Could you check a few things on this model? Use its own coordinates, in mm. Give positions to 0.01 mm unless a question says otherwise; leave off trailing zeros. Order: outer loops, then holes, each group sorted by start corner. A loop starts at its lowest first (then second) coordinate and runs counter-clockwise, first axis right, second up.
(1) If I drill on probe 1 along Y at (x, z) = (48, 4); probe 2 along X at (y, z) = (3, 2); probe 3 along Y at (x, z) = (-51, 0.75), over which ranges is the centre line in solid material (lowest first)?
(2) Imagine slicing it at A-A, the plane x = 48. Write out the boundary of the cut face in (y, z).
(3) Imagine slicing it at C-C, the plane z = 2.25. Write out the boundary of the cut face in (x, y).
(4) Will this pin go through, and if not, where does the flat tip stop? pin 1 (10 mm diameter, centred on x = 48, y = 0, fed in from +Z).
(5) If we mould it in two halves opening along Y, with no side actions, what happens to faces 1 (the cylindrical face through (73, 19, 6)), 2 (the flat face through (-1, 0, 12)), 3 (the cylindrical face through (42.505, -0.242, 6.084)), 4 (the flat face through (-1, -20, 6))? For each: released by +Y, released by -Y, zero draft, split by the parting line, or undercut.
(6) Imagine slicing it at B-B, the plane y = 0. Write out the boundary of the cut face in (x, z).
from build123d import *

# Parameters (mm, degrees)
SKETCH1_W           = 150
SKETCH1_H           = 40
BOSS_EXTRUDE1_DEPTH = 12
SKETCH2_R           = 5.5
CUT_EXTRUDE1_DEPTH  = 8
FILLET1_R           = 5
CUT_EXTRUDE2_START  = -12
SKETCH3_R           = 5.5
CUT_EXTRUDE2_DEPTH  = 12


with BuildPart() as part:
    # Sketch1 → Boss-Extrude1 (new body)
    with BuildSketch(Plane.XY):
        Rectangle(SKETCH1_W, SKETCH1_H)
    extrude(amount=BOSS_EXTRUDE1_DEPTH)

    # Sketch2 → Cut-Extrude1 (cut)
    with BuildSketch(Plane.XY.offset(12)):
        with Locations((-48, 0)):
            Circle(SKETCH2_R)
        with Locations((48, 0)):
            Circle(SKETCH2_R)
    extrude(amount=-CUT_EXTRUDE1_DEPTH, mode=Mode.SUBTRACT)

    # Fillet1
    fillet1_edges = [part.edges().sort_by_distance(p)[0] for p in [
        (75, -20, 6),
        (-75, -20, 6),
        (-75, 20, 6),
        (75, 20, 6),
    ]]
    fillet(fillet1_edges, radius=FILLET1_R)

    # Sketch3 → Cut-Extrude2 (cut)
    with BuildSketch(Plane(origin=(0, 0, 0), x_dir=(-1, 0, 0), z_dir=(0, 0, -1)).offset(CUT_EXTRUDE2_START)):
        with Locations(Location((-48, 0, 0), (0, 0, 180))):
            Circle(SKETCH3_R)
        with Locations(Location((48, 0, 0), (0, 0, 180))):
            Circle(SKETCH3_R)
    extrude(amount=CUT_EXTRUDE2_DEPTH, mode=Mode.SUBTRACT)


solid = part.part
Answer block:
1. probe 1: y = -20 to -5.5, 5.5 to 20
1. probe 2: x = -75 to -52.61, -43.39 to 43.39, 52.61 to 75
1. probe 3: y = -20 to -4.61, 4.61 to 20
2. outline: (-20, 0) - (-5.5, 0) - (-5.5, 12) - (-20, 12) - close; (5.5, 0) - (20, 0) - (20, 12) - (5.5, 12) - close
3. outline: (-75, -15) arc R5 ccw to (-70, -20) - (70, -20) arc R5 ccw to (75, -15) - (75, 15) arc R5 ccw to (70, 20) - (-70, 20) arc R5 ccw to (-75, 15) - close; hole circle Ø11 at (-48, 0); hole circle Ø11 at (48, 0)
4. pin 1: passes through
5. face 1: released by +Y
5. face 2: zero draft
5. face 3: undercut
5. face 4: released by -Y
6. outline: (-75, 0) - (-53.5, 0) - (-53.5, 12) - (-75, 12) - close; (-42.5, 0) - (42.5, 0) - (42.5, 12) - (-42.5, 12) - close; (53.5, 0) - (75, 0) - (75, 12) - (53.5, 12) - close
